Read the model definition and answer for the solid it produces. Units are mm, in the model's axes. Face numbers are marked on the shaded views. A direction names the side the tool comes from. Give positions to 0.01 mm unless a question says otherwise; leave off trailing zeros. Order: outer loops, then holes, each group sorted by start corner. A loop starts at its lowest first (then second) coordinate and runs counter-clockwise, first axis right, second up. Notation, with made-up numbers: (63.25, -39.5) -> (106.25, -39.5) arc R28 cw to (106.25, -15.5) -> close; hole circle Ø7 at (46.5, 43.5). An arc over 180 degrees is marked (long way). Use one line per item in the form item = value.
```python
from build123d import *

# Parameters (mm, degrees)
EXTRUDE_1_DEPTH     = 4.5
SKETCH_4_R          = 13.05
EXTRUDE_3_DEPTH     = 17
CUT_EXTRUDE_2_REACH = 49.689
SKETCH_5_R          = 9
CHAMFER_1_SIZE      = 1


with BuildPart() as part:
    # 草图1 → 凸台-拉伸1 (new, symmetric)
    with BuildSketch(Plane.XY):
        Polygon((15.588457268, 0), (7.794228634, 13.5), (-7.794228634, 13.5), (-15.588457268, 0), (-7.794228634, -13.5), (7.794228634, -13.5), align=None)
    extrude(amount=EXTRUDE_1_DEPTH, both=True)

    # 草图4 → 凸台-拉伸3 (add)
    with BuildSketch(Plane(origin=(0, 0, -4.5), x_dir=(-1, 0, 0), z_dir=(0, 0, -1))):
        Circle(SKETCH_4_R)
    extrude_3 = extrude(amount=EXTRUDE_3_DEPTH)

    # 镜向1: 凸台-拉伸3 across plane
    add(extrude_3.mirror(Plane.XY))

    # 草图5 → 切除-拉伸2 (cut, up to next)
    with BuildSketch(Plane(origin=(0, 0, -21.5), x_dir=(-1, 0, 0), z_dir=(0, 0, -1)), mode=Mode.PRIVATE) as cut_extrude_2_sk1:
        Circle(SKETCH_5_R)
    cut_extrude_2_tool1 = extrude(cut_extrude_2_sk1.sketch, amount=-CUT_EXTRUDE_2_REACH, mode=Mode.PRIVATE) & part.part
    add(cut_extrude_2_tool1.solids().sort_by_distance((0, 0, -21.5))[0], mode=Mode.SUBTRACT)

    # 倒角1
    chamfer_1_edges = [part.edges().sort_by_distance(p)[0] for p in [
        (13.05, 0, -21.5),
        (13.05, 0, 21.5),
    ]]
    chamfer(chamfer_1_edges, length=CHAMFER_1_SIZE)


solid = part.part
```
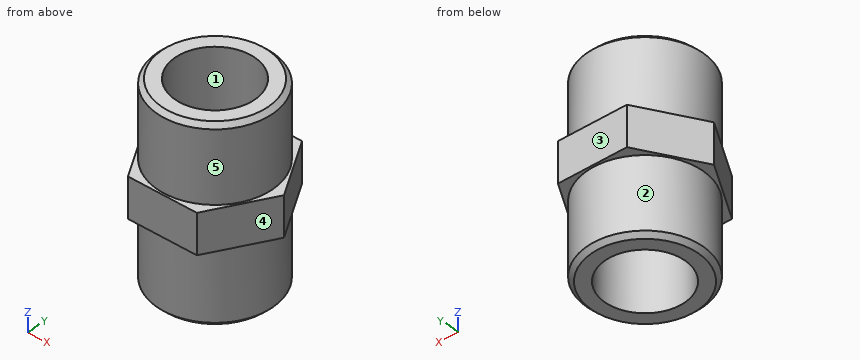
Item 1: Straight lines are drawn through the part: L1, parallel to Y at x = 0, z = 6; L2, parallel to Y at x = 0, z = 1; L3, parallel to Z at x = 8, y = 12. For each, find the intervals that lie inside material, in ascending order. Write a range as from..to.
Checks:
L1 = -13.05..-9, 9..13.05
L2 = -13.5..-9, 9..13.5
L3 = -4.5..4.5
Item 2: Determine the mould class of the marked faces 1, 2 and 3 for opening direction Y: +Y half, -Y half, draft (parallel to the pull), parting line (faces both ways), or undercut.
Checks:
face_1 = undercut
face_2 = parting line
face_3 = +Y half
Item 3: Given pin 1 Ø1 at (y, z) = (2, -0.5) entering from -X; pin 2 Ø6 at (y, z) = (-5, 3) entering from -X; pin 3 Ø5 at (x, z) = (11.5, 12) entering from +Y; pin 4 Ø3 at (x, y) = (12, 10.5) entering from +Z, each flat-ended and moving along its own axis, determine where each tip first touches the part or whether it passes through.
Checks:
pin_1 = -14.72
pin_2 = -14.43
pin_3 = 9.45
pin_4 = through
Item 4: Which of the six approach directions +Z, -Z, +X, -X, +Y, -Y give full straight-line access (tool end or side, diameter ignored) to the marked faces 4 and 5?
Checks:
face_4 = +Z, -Z, +X, -Y
face_5 = +Z
Item 5: The part is cut by section B-B on z = 6. Give the vertices of the cut face in (x, y), and give its area (3 significant figures).
Checks:
outline = circle Ø26.1 at (0, 0); hole circle Ø18 at (0, 0)
area = 281 mm²
Item 6: The part is cut by section A-A on x = 0. Give the vertices of the cut face in (y, z), and give its area (3 significant figures).
Checks:
outline = (-13.5, -4.5) -> (-13.05, -4.5) -> (-13.05, -20.5) -> (-12.05, -21.5) -> (-9, -21.5) -> (-9, 21.5) -> (-12.05, 21.5) -> (-13.05, 20.5) -> (-13.05, 4.5) -> (-13.5, 4.5) -> close; (9, -21.5) -> (12.05, -21.5) -> (13.05, -20.5) -> (13.05, -4.5) -> (13.5, -4.5) -> (13.5, 4.5) -> (13.05, 4.5) -> (13.05, 20.5) -> (12.05, 21.5) -> (9, 21.5) -> close
area = 354 mm²
